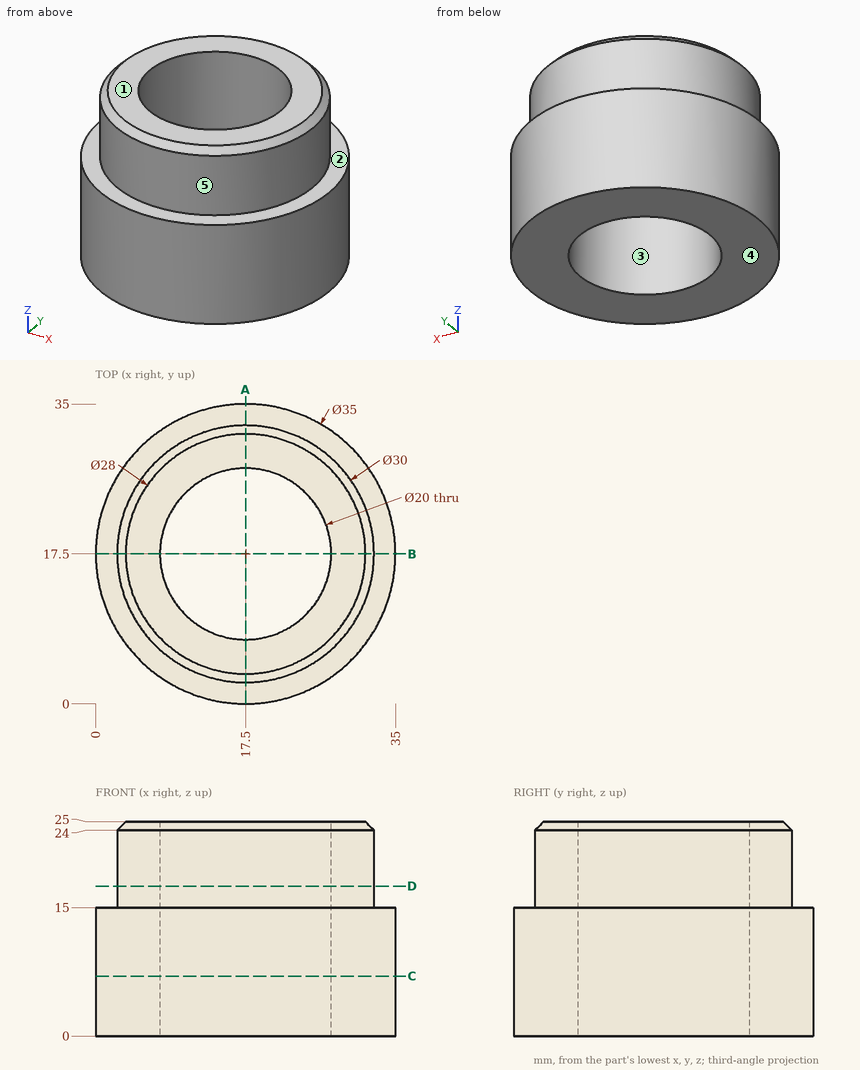
Geometry: see drawing. Coordinates: mm, zero at the bounding-box minimum. A direction names the side the tool comes from. Coordinates: 2 decimals unless noted, no trailing zeros. Loops run counter-clockwise (first coordinate to the right, second up) from the corner with the lowest first, then second, coordinate; pieces in that order, holes last. Notation, with made-up numbers: (78, -27) - (125, -27) arc R24 ccw to (125, 5) - close; hole circle Ø7 at (-19.75, 14.5). An arc over 180 degrees is marked (long way). Return JSON: item names as keys, results as strings.
Q1. Section D-D, the plane z = 17.5. Return loops of the section in (x, y), plus the area to 3 significant figures.
Results:
{"outline": "circle Ø30 at (17.5, 17.5); hole circle Ø20 at (17.5, 17.5)", "area": "393 mm2"}
Q2. Section C-C, the plane z = 7. Return loops of the section in (x, y).
Results:
{"outline": "circle Ø35 at (17.5, 17.5); hole circle Ø20 at (17.5, 17.5)"}
Q3. Access query for the marked faces 1 and 2. Directions: +Z, -Z, +X, -X, +Y, -Y. A direction counts if a zero-diameter tool reaches every point of the face in a straight line with its end or side. Return the directions, or none.
Results:
{"face 1": "+Z, +X, -X, +Y, -Y", "face 2": "+Z"}
Q4. Contact query for flat-ended pins moving along their axis: P1, Ø2, axis at y = 28.5, z = 11, coming from the +X side; P2, Ø8, axis at y = 28.5, z = 12, coming from the -X side; P3, Ø4, axis at y = 28.5, z = 22, coming from the -X side. Output: stop coordinate, or through.
Results:
{"P1": "x = 31.86", "P2": "x = 1.46", "P3": "x = 5.5"}
Q5. Section A-A, the plane x = 17.5. Return loops of the section in (y, z).
Results:
{"outline": "(0, 0) - (7.5, 0) - (7.5, 25) - (3.5, 25) - (2.5, 24) - (2.5, 15) - (0, 15) - close; (27.5, 0) - (35, 0) - (35, 15) - (32.5, 15) - (32.5, 24) - (31.5, 25) - (27.5, 25) - close"}
Q6. Material intervals for line 1 along Y through (x, z) = (17.5, 17); line 2 along Y through (x, z) = (17.5, 5.5); line 3 along X through (y, z) = (14, 10.5), sorted ascending.
Results:
{"line 1": "2.5 to 7.5, 27.5 to 32.5", "line 2": "0 to 7.5, 27.5 to 35", "line 3": "0.35 to 8.13, 26.87 to 34.65"}
Q7. Mould query, pull axis X, two halves, no side actions, for the marked faces 3, 4 and 5. Classes: released by +X, released by -X, zero draft, split by the parting line, or undercut.
Results:
{"face 3": "undercut", "face 4": "zero draft", "face 5": "split by the parting line"}
